Here's how the part is built. I have some questions about the finished solid (model axes, mm). Give positions to 0.01 mm unless a question says otherwise; leave off trailing zeros. Write each loop counter-clockwise with the first axis right and the second up, starting at its lowest first coordinate (ties: lowest second). Pieces come first, ordered by that corner, then holes. Notation, with made-up numbers: (-37, 25.25) - (17, 25.25) arc R13 ccw to (17, 37.25) - close; hole circle Ø3 at (81.25, -16). An arc over 180 degrees is marked (long way). Use a Markdown table: item, result.
```python
from build123d import *

# Parameters (mm, degrees)
RING_OUTLINE_SKETCH_132_R = 66
RING_DISC_132X5_DEPTH     = 5
WINDOW_CUT_DEPTH          = 25
WINDOW_PATTERN_10X_COUNT  = 10
BORE_SKETCH_80_R          = 40
CENTRE_BORE_80_DEPTH      = 25


with BuildPart() as part:
    # Ring Outline Sketch Ø132 → Ring Disc Ø132x5 (new body)
    with BuildSketch(Plane.XY):
        Circle(RING_OUTLINE_SKETCH_132_R)
    extrude(amount=RING_DISC_132X5_DEPTH)

    # Window Sketch → Window Cut (cut)
    with BuildSketch(Plane.XY.offset(5)):
        with BuildLine():
            Line((5, 49.749371855), (5, 57.92236183))
            ThreePointArc((5, 57.92236183), (4.450326955, 59.299515316), (3.103448276, 59.919684652))
            ThreePointArc((3.103448276, 59.919684652), (0, 60), (-3.103448276, 59.919684652))
            ThreePointArc((-3.103448276, 59.919684652), (-4.450326955, 59.299515316), (-5, 57.92236183))
            Line((-5, 57.92236183), (-5, 49.749371855))
            ThreePointArc((-5, 49.749371855), (0, 50), (5, 49.749371855))
        make_face()
    window_cut = extrude(amount=-WINDOW_CUT_DEPTH, mode=Mode.SUBTRACT)

    # Window Pattern 10x: Window Cut ×10 about axis
    window_pattern_10x_axis = Axis((0, 0, 0), (0, 0, 1))
    for i in range(1, WINDOW_PATTERN_10X_COUNT):
        add(window_cut.rotate(window_pattern_10x_axis, i * 360 / WINDOW_PATTERN_10X_COUNT), mode=Mode.SUBTRACT)

    # Bore Sketch Ø80 → Centre Bore Ø80 (cut)
    with BuildSketch(Plane.XY.offset(5)):
        Circle(BORE_SKETCH_80_R)
    extrude(amount=-CENTRE_BORE_80_DEPTH, mode=Mode.SUBTRACT)


solid = part.part
```
Item 1: Will this pin go through, and if not, where does the flat tip stop? pin 1 Ø2 at (x, z) = (6, 3) entering from -Y.
Values:
| item | result |
|---|---|
| pin 1 | stops at y = -65.81 |
Item 2: If we section it at D-D, the plane z = 2.45: Count the separate pieces of the cut face and the enclosed holes in it, plus the area to 3 significant figures.
Values:
| item | result |
|---|---|
| separate pieces | 1 |
| enclosed holes | 11 |
| area | 7,670 mm2 |
Item 3: I need wall thicknesses on line 1 along Y through (x, z) = (0, 2.35); line 2 along Y through (x, z) = (53, 1.85); line 3 along X through (y, z) = (-47, 4.2). Which ranges of each line are inside material? Lowest first, please. Write a range as [from, to].
Values:
| item | result |
|---|---|
| line 1 | y = [-66, -60], [-50, -40], [40, 50], [60, 66] |
| line 2 | y = [-39.33, -22.48], [-11.96, 11.96], [22.48, 39.33] |
| line 3 | x = [-46.34, -37.3], [-27.97, 27.97], [37.3, 46.34] |
Item 4: If we section it at A-A, the plane y = 0: Write out the boundary of the cut face in (x, z).
Values:
| item | result |
|---|---|
| outline | (-66, 0) - (-40, 0) - (-40, 5) - (-66, 5) - close; (40, 0) - (66, 0) - (66, 5) - (40, 5) - close |
Item 5: If we section it at B-B, the plane x = 0: Write out the boundary of the cut face in (y, z).
Values:
| item | result |
|---|---|
| outline | (-66, 0) - (-60, 0) - (-60, 5) - (-66, 5) - close; (-50, 0) - (-40, 0) - (-40, 5) - (-50, 5) - close; (40, 0) - (50, 0) - (50, 5) - (40, 5) - close; (60, 0) - (66, 0) - (66, 5) - (60, 5) - close |
Item 6: Thinking about a two-plate mould opening in X: for faces 1 (the cylindrical face through (35.23, -48.57, 2.54)), 2 (the cylindrical face through (60.967, -25.278, 2.465)), 3 (the flat face through (28.4, -28.4, 5)), which applies, +X half, -X half, draft (parallel to the pull), parting line (faces both ways), or undercut?
Values:
| item | result |
|---|---|
| face 1 | undercut |
| face 2 | parting line |
| face 3 | draft |
Item 7: If we section it at C-C, the plane x = 21: Write out the boundary of the cut face in (y, z).
Values:
| item | result |
|---|---|
| outline | (-62.57, 0) - (-34.04, 0) - (-34.04, 5) - (-62.57, 5) - close; (34.04, 0) - (62.57, 0) - (62.57, 5) - (34.04, 5) - close |
